The listing builds one solid part. Answer for the finished solid, in the listing's coordinates (mm). Face numbers are marked on the shaded views. A direction names the side the tool comes from. Coordinates: 2 decimals unless noted, no trailing zeros. Order: outer loops, then holes, each group sorted by start corner. A loop starts at its lowest first (then second) coordinate and runs counter-clockwise, first axis right, second up. Notation, with made-up numbers: M 20.5,4 L 62.5,4 A16 cw 62.5,29 Z; hole C 69.25,89 d2. An arc over 180 degrees is marked long. One line per item, written item: value. Start each with the question number.
Q1. The part is cut by section A-A on z = 7. Give the vertices of the cut face in (x, y), then the cut area to 4 significant figures.
Q2. Straight lines are drawn through the part: line 1 along Y through (x, z) = (17.5, 14.5); line 2 along Y through (x, z) = (30, 5.25). For each, find the intervals that lie inside material, in ascending order. Write a range as [from, to].
Q3. The part is cut by section D-D on z = 13.75. Give the vertices of the cut face in (x, y), then the cut area to 3 significant figures.
Q4. Each of these flat-tipped pins is pushed along its axis until it touches: pin 1 Ø2 at (y, z) = (-20.5, 3.5) entering from -X; pin 2 Ø3 at (x, y) = (13.5, 3) entering from -Z; pin 3 Ø4 at (x, y) = (25, 3.5) entering from -Z; pin 4 Ø5 at (x, y) = (23, 5) entering from +Z. Where does it stop, or does it pass through?
Q5. The part is cut by section B-B on x = 28.5. Give the vertices of the cut face in (y, z), then the cut area to 3 significant figures.
Q6. For the marked faces 1, 2, 3, 4 and 5, determine the directions among +Z, -Z, +X, -X, +Y, -Y from which every point of the face is accessible in a straight line to the end or side of a thin tool.
Q7. The part is cut by section C-C on x = 7.5. Give the vertices of the cut face in (y, z), then the cut area to 3 significant figures.
```python
from build123d import *

# Parameters (mm, degrees)
SKETCH1_W           = 40
SKETCH1_H           = 30
BOSS_EXTRUDE1_DEPTH = 18
BOSS_EXTRUDE3_START = 5
BOSS_EXTRUDE3_DEPTH = 5


with BuildPart() as part:
    # Sketch1 → Boss-Extrude1 (new body)
    with BuildSketch(Plane.XY):
        with Locations((20, -15)):
            Rectangle(SKETCH1_W, SKETCH1_H)
    extrude(amount=BOSS_EXTRUDE1_DEPTH)

    # Sketch2 → Boss-Extrude3 (add)
    with BuildSketch(Plane.XY.offset(BOSS_EXTRUDE3_START)):
        Polygon((17.5, 10), (17.5, 2), (5, 0), (35, 0), (22.5, 2), (22.5, 10), align=None)
    extrude(amount=BOSS_EXTRUDE3_DEPTH)


solid = part.part
```
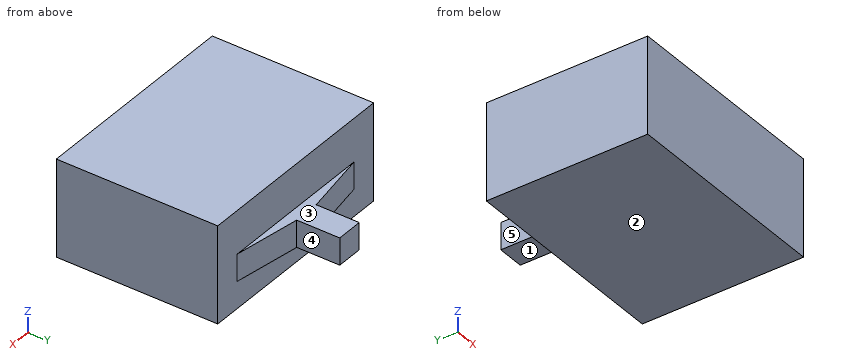
Output:
1. outline: M 0,-30 L 40,-30 L 40,0 L 35,0 L 22.5,2 L 22.5,10 L 17.5,10 L 17.5,2 L 5,0 L 0,0 Z
1. area: 1,275 mm^2
2. line 1: y = [-30, 0]
2. line 2: y = [-30, 0.8]
3. outline: M 0,-30 L 40,-30 L 40,0 L 0,0 Z
3. area: 1,200 mm^2
4. pin 1: stops at x = 0
4. pin 2: passes through
4. pin 3: stops at z = 5
4. pin 4: stops at z = 10
5. outline: M -30,0 L 0,0 L 0,5 L 1.04,5 L 1.04,10 L 0,10 L 0,18 L -30,18 Z
5. area: 545 mm^2
6. face 1: -Z, +X, -X, +Y
6. face 2: -Z, +X, -X, +Y, -Y
6. face 3: +Z, +X, -X, +Y
6. face 4: +Z, -Z, +X, +Y
6. face 5: +Z, -Z, -X, +Y
7. outline: M -30,0 L 0,0 L 0,5 L 0.4,5 L 0.4,10 L 0,10 L 0,18 L -30,18 Z
7. area: 542 mm^2
